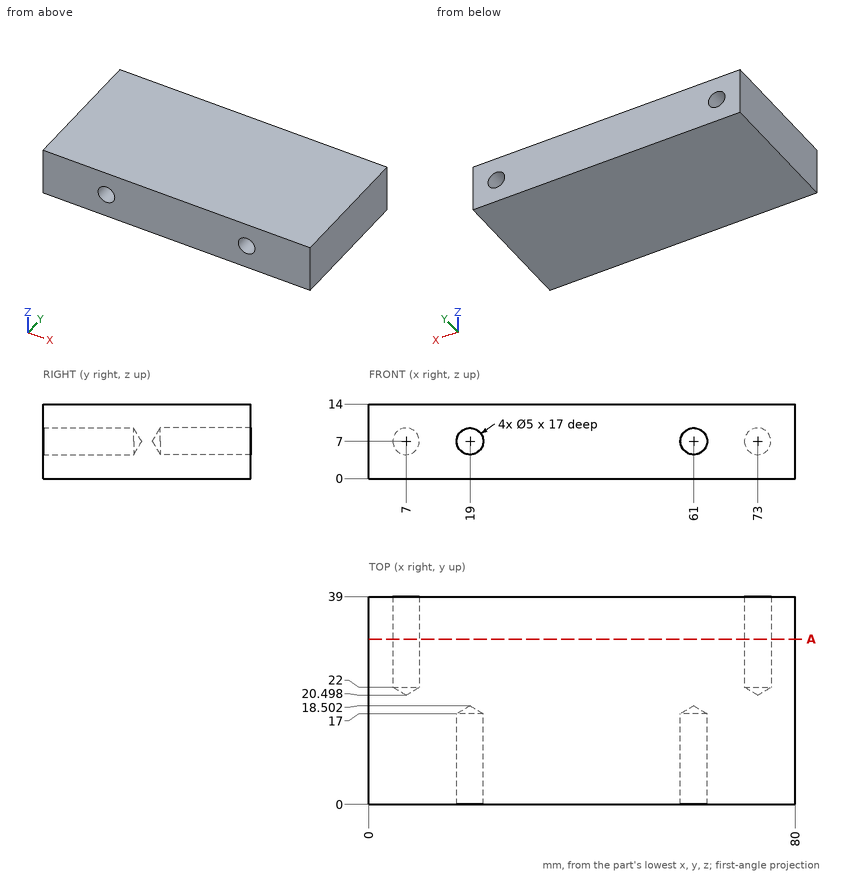
Design review of the part shown in the three views and the two pictorial views. Dimensions are in mm from the part's minimum x, y and z. Give positions to 0.01 mm unless a question says otherwise; leave off trailing zeros. Loops run counter-clockwise (first coordinate to the right, second up) from the corner with the lowest first, then second, coordinate; pieces in that order, holes last. Notation, with made-up numbers: (77.5, -17.5) - (136.5, -17.5) arc R9 ccw to (136.5, -11.5) - close; hole circle Ø7 at (-28, 24.5). An arc over 180 degrees is marked (long way). Write item = value, one per line.
1) Take a section at A-A on y = 31. State the section outline as (x, z) points.
Result sheet:
outline = (0, 0) - (80, 0) - (80, 14) - (0, 14) - close; hole circle Ø5 at (7, 7); hole circle Ø5 at (73, 7)
2) To check wall thickness, follow line 1 (Z direction, x = 61, y = 11.25); line 2 (X direction, y = 2, z = 6); line 3 (X direction, y = 13, z = 6.25) (1 decimal). State the ranges of each line that lie inside material, in increasing order.
Result sheet:
line_1 = 0 to 4.5, 9.5 to 14
line_2 = 0 to 16.71, 21.29 to 58.71, 63.29 to 80
line_3 = 0 to 16.6, 21.4 to 58.6, 63.4 to 80
3) Clearance check with flat-ended pins moving along their axes: pin 1 Ø6 at (x, z) = (27, 10) entering from -Y; pin 2 Ø4 at (x, z) = (73, 7) entering from +Y. State where each tip first meets the part, or that it passes through.
Result sheet:
pin_1 = 0
pin_2 = 21.7
